from build123d import *

# Parameters (mm, degrees)
BASEHEAD_DEPTH  = 3.65
SKETCH3_R       = 2.5
BASEBODY_DEPTH  = 30
CHAMFER1_SIZE   = 0.433
SLOT_DEPTH      = 35.663103343
SLOT_DEPTH_BACK = 35.663103343
SKETCH5_W       = 1.2
SKETCH5_H       = 1.2


with BuildPart() as part:
    # Sketch-BaseHead → BaseHead (new body)
    with BuildSketch(Plane(origin=(0, 0, 0), x_dir=(0, 0, -1), z_dir=(1, 0, 0))):
        Polygon((2.245892547, -3.89), (4.491785094, 0), (2.245892547, 3.89), (-2.245892547, 3.89), (-4.491785094, 0), (-2.245892547, -3.89), align=None)
    extrude(amount=BASEHEAD_DEPTH)

    # Sketch1 → Revolve1 (revolve)
    with BuildSketch(Plane.XY, mode=Mode.PRIVATE) as revolve1_sk:
        Polygon((3.65, 0), (4.15, 0), (4.15, -3.44), (3.65, -3.89), align=None)
    revolve(revolve1_sk.sketch.rotate(Axis((-4.001564945, 0, 0), (1, 0, 0)), 270), axis=Axis((-4.001564945, 0, 0), (1, 0, 0)))

    # Sketch3 → BaseBody (add)
    with BuildSketch(Plane(origin=(4.15, 0, 0), x_dir=(0, 0, -1), z_dir=(1, 0, 0))):
        Circle(SKETCH3_R)
    extrude(amount=BASEBODY_DEPTH)

    # Chamfer1
    chamfer1_edges = [part.edges().sort_by_distance(p)[0] for p in [
        (34.15, 0, 2.5),
    ]]
    chamfer(chamfer1_edges, length=CHAMFER1_SIZE)

    # Sketch4 → HeadChamfer (revolve, cut)
    with BuildSketch(Plane(origin=(-0.264637255, 0, 5.916896391), x_dir=(0, 0, -1), z_dir=(0, 1, 0)), mode=Mode.PRIVATE) as headchamfer_sk:
        Polygon((10.408681485, -0.264637255), (9.806896391, -0.264637255), (10.408681485, -0.483669117), align=None)
    revolve(headchamfer_sk.sketch.rotate(Axis((-4.001564945, 0, 0), (1, 0, 0)), 180), axis=Axis((-4.001564945, 0, 0), (1, 0, 0)), mode=Mode.SUBTRACT)

    # Sketch5 → Slot (cut, two sides: drawn at the far end of the back side and taken through both)
    with BuildSketch(Plane(origin=(0, 0, 0), x_dir=(1, 0, 0), z_dir=(0, 1, 0)).offset(-SLOT_DEPTH_BACK)):
        with Locations((0.6, 0)):
            Rectangle(SKETCH5_W, SKETCH5_H)
    extrude(amount=SLOT_DEPTH + SLOT_DEPTH_BACK, mode=Mode.SUBTRACT)


solid = part.part
Read the model definition and answer for the solid it produces. Units are mm, in the model's axes. A direction names the side the tool comes from. Round coordinates to 2 decimals unless told otherwise and drop trailing zeros. Write each loop counter-clockwise with the first axis right and the second up, starting at its lowest first coordinate (ties: lowest second). Pieces come first, ordered by that corner, then holes.
1. The part is cut by section A-A, the plane x = 20. Determine the outline of the cut face in (y, z).
2. Determine the mould class of faces 6 (the face through (1, 0, 0.6)), 7 (the face through (0.06, 3.55, -1.97)), 8 (the face through (0, 0, -2)) for opening direction Z: pulls with the +Z half, pulls with the -Z half, needs draft (parallel to the pull), parting line crosses it, or undercut.
3. Which of the six approach directions +Z, -Z, +X, -X, +Y, -Y give full straight-line access (tool end or side, diameter ignored) to faces 1 (the face through (34.15, 0, 0)), 2 (the face through (2, -3.89, 0)), 3 (the face through (1.2, 0, 0)), 4 (the face through (3.65, 0, -4.1)), 5 (the face through (4.15, 3, 0))?
4. Given pin 1 Ø0.6 at (y, z) = (-3, -1.5) entering from +X; pin 2 Ø2 at (x, y) = (25, -1) entering from -Z; pin 3 Ø1 at (y, z) = (0, 0) entering from -X, each flat-ended and moving along its own axis, determine where each tip first touches the part or whether it passes through.
5. Straight lines are drawn through the part: L1, parallel to X at y = 1.5, z = 2.75; L2, parallel to X at y = -1.5, z = -0.25; L3, parallel to Y at x = 20, z = 0. For each, find the intervals that lie inside material, in ascending order.
Values:
1. outline: circle Ø5 at (0, 0)
2. face 6: undercut
2. face 7: pulls with the -Z half
2. face 8: needs draft
3. face 1: +Z, -Z, +X, +Y, -Y
3. face 2: +Z, -Z, +X, -X, -Y
3. face 3: -X, +Y, -Y
3. face 4: -Z, +X
3. face 5: +X
4. pin 1: stops at x = 4.15
4. pin 2: stops at z = -2.5
4. pin 3: stops at x = 1.2
5. L1: x = 0 to 4.15
5. L2: x = 1.2 to 34.15
5. L3: y = -2.5 to 2.5
